Model file for the job. Use its own axes, mm. A direction names the side the tool comes from. Give positions to 0.01 mm unless a question says otherwise; leave off trailing zeros. Loops run counter-clockwise (first coordinate to the right, second up) from the corner with the lowest first, then second, coordinate; pieces in that order, holes last. Notation, with made-up numbers: M 0.25,-8 L 42.25,-8 A20 cw 42.25,5 Z; hole C -25,53 d7. An arc over 180 degrees is marked long. Answer in a Markdown table with one row per item.
```python
from build123d import *

# Parameters (mm, degrees)
L_BRACKET_BODY_DEPTH = 20
CLAMP_BORE_SKETCH_R  = 4
CLAMP_BORE_DEPTH     = 52.46843693
CLAMP_SLIT_DEPTH     = 52.46843693
CLEVIS_LUG_SKETCH_R  = 3
CLEVIS_LUG_DEPTH     = 5
LUG_PIN_HOLE_DEPTH   = 12


with BuildPart() as part:
    # Bracket Profile Sketch → L-Bracket Body (new body)
    with BuildSketch(Plane.XY):
        Polygon((0, 0), (55, 0), (55, 10), (20, 10), (20, 32), (0, 32), align=None)
    extrude(amount=L_BRACKET_BODY_DEPTH)

    # Clamp Bore Sketch → Clamp Bore (cut, through all)
    with BuildSketch(Plane(origin=(20, 0, 0), x_dir=(0, 0, -1), z_dir=(1, 0, 0))):
        with Locations((-10, 18)):
            Circle(CLAMP_BORE_SKETCH_R)
    extrude(amount=-CLAMP_BORE_DEPTH, mode=Mode.SUBTRACT)

    # Clamp Slit Sketch → Clamp Slit (cut, through all)
    with BuildSketch(Plane(origin=(20, 0, 0), x_dir=(0, 0, -1), z_dir=(1, 0, 0))):
        with BuildLine():
            ThreePointArc((-11, 21.872983346), (-10, 22), (-9, 21.872983346))
            Line((-9, 21.872983346), (-9, 32))
            Line((-9, 32), (-11, 32))
            Line((-11, 32), (-11, 21.872983346))
        make_face()
    extrude(amount=-CLAMP_SLIT_DEPTH, mode=Mode.SUBTRACT)

    # Clevis Lug Sketch → Clevis Lug (add)
    with BuildSketch(Plane(origin=(0, 10, 0), x_dir=(1, 0, 0), z_dir=(0, 1, 0))):
        with BuildLine():
            Line((39.847164106, -12.116295981), (40, -20))
            Line((40, -20), (51.846036937, -20))
            Line((51.846036937, -20), (51.846036937, -12))
            ThreePointArc((51.846036937, -12), (45.787886215, -6.000281799), (39.847164106, -12.116295981))
        make_face()
        with Locations(Location((45.846036937, -12, 0), (0, 0, 270))):
            Circle(CLEVIS_LUG_SKETCH_R, mode=Mode.SUBTRACT)
    extrude(amount=CLEVIS_LUG_DEPTH)

    # Lug Pin Hole Sketch → Lug Pin Hole (cut)
    with BuildSketch(Plane(origin=(51.846036937, 0, 0), x_dir=(0, 0, -1), z_dir=(1, 0, 0))):
        Polygon((-20, 15), (-20, 10), (-6, 15), align=None)
    extrude(amount=-LUG_PIN_HOLE_DEPTH, mode=Mode.SUBTRACT)


solid = part.part
```
Q1. Drop flat-ended pins along their axis: pin 1 (3 mm diameter, centred on y = 24.5, z = 10.5, fed in from +X); pin 2 (3 mm diameter, centred on y = 12, z = 14.5, fed in from +X); pin 3 (1.8 mm diameter, centred on x = 45.5, z = 13, fed in from +Y); pin 4 (1 mm diameter, centred on x = 40, y = 15.5, fed in from -Z). Give the stop position or say it passes through.
Reported:
| item | result |
|---|---|
| pin 1 | x = 20 |
| pin 2 | x = 51.85 |
| pin 3 | y = 10 |
| pin 4 | through |
Q2. Saw through at A-A (y = 18). Give the cut face in (x, z), and give its area (3 significant figures).
Reported:
| item | result |
|---|---|
| outline | M 0,0 L 20,0 L 20,6 L 0,6 Z; M 0,14 L 20,14 L 20,20 L 0,20 Z |
| area | 240 mm² |
Q3. Mould opens along X. For faces 5 (the face through (27, 0, 10)), 6 (the face through (45.978, 11.539, 9.003)), 7 (the face through (55, 5, 10)) say: released by +X, released by -X, zero draft, split by the parting line, or undercut.
Reported:
| item | result |
|---|---|
| face 5 | zero draft |
| face 6 | undercut |
| face 7 | released by +X |
Q4. Saw through at B-B (x = 3.5). Give the cut face in (y, z).
Reported:
| item | result |
|---|---|
| outline | M 0,0 L 32,0 L 32,9 L 21.87,9 A4 cw long 21.87,11 L 32,11 L 32,20 L 0,20 Z |
Q5. Probe probe 1 along Z at (x, y) = (8, 18); probe 2 along X at (y, z) = (11.9, 12); probe 3 along Z at (x, y) = (10.5, 28). List the from-to ranges inside material, lowest first.
Reported:
| item | result |
|---|---|
| probe 1 | 0 to 6, 14 to 20 |
| probe 2 | 0 to 20, 39.85 to 42.85, 48.85 to 51.85 |
| probe 3 | 0 to 9, 11 to 20 |
Q6. 3-axis set-ups, long thin cutter, end or side, ignore diameter. For faces 1 (the face through (10, 27, 11)), 2 (the face through (51.846, 11, 14)), 3 (the face through (45.93, 11.354, 16.209)), 4 (the face through (46, 10, 12)): which of +Z, -Z, +X, -X, +Y, -Y reach the whole face in a straight line?
Reported:
| item | result |
|---|---|
| face 1 | +X, -X, +Y |
| face 2 | +Z, -Z, +X, +Y |
| face 3 | +Z, +X, +Y |
| face 4 | +Y |
Q7. Saw through at D-D (z = 18.5). Give the cut face in (x, y).
Reported:
| item | result |
|---|---|
| outline | M 0,0 L 55,0 L 55,10 L 51.85,10 L 51.85,10.54 L 39.97,10.54 L 39.97,10 L 20,10 L 20,32 L 0,32 Z |
Q8. Saw through at C-C (z = 2.5). Give the cut face in (x, y), and give its area (3 significant figures).
Reported:
| item | result |
|---|---|
| outline | M 0,0 L 55,0 L 55,10 L 20,10 L 20,32 L 0,32 Z |
| area | 990 mm² |
